Input: dimensioned drawing with shaded views. Units: mm. Origin: part minimum x, y, z. Round coordinates to 2 decimals unless told otherwise and drop trailing zeros. Loops run counter-clockwise (first coordinate to the right, second up) from the corner with the lowest first, then second, coordinate; pieces in that order, holes last. Notation, with made-up numbers: (-33.75, -26.75) - (-1.75, -26.75) arc R19 ccw to (-1.75, -12.75) - close; hole circle Ø7 at (62.25, 61.5). An arc over 180 degrees is marked (long way). Write each question's results on one line, items separated by ' | '.
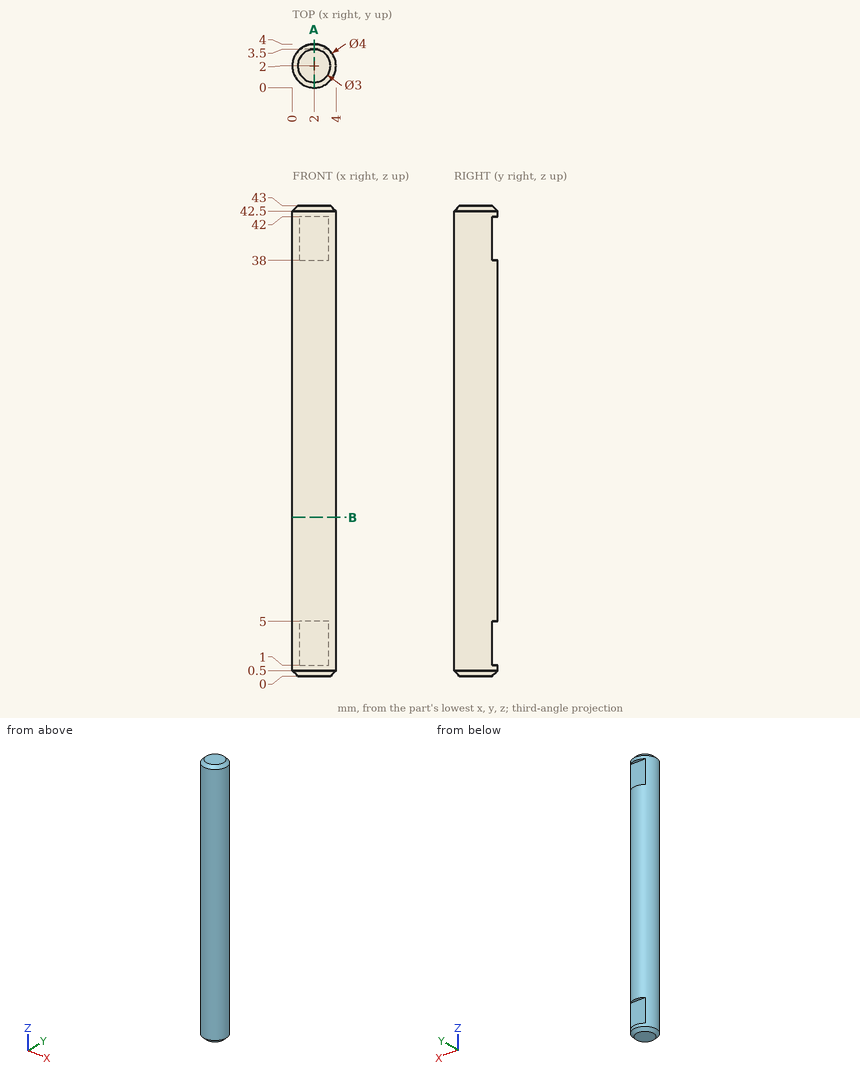
1. Line query: line 1 (Y direction, x = 2.1, z = 4); line 2 (X direction, y = 1.9, z = 32.5); line 3 (X direction, y = 1.1, z = 20). Output: solid intervals per line, ascending. Write a range as [from, to].
Answer:
line 1: [0, 3.5] | line 2: [0, 4] | line 3: [0.21, 3.79]
2. Contact query for a flat-ended pin moving along its axis: pin 1 (1.5 mm diameter, centred on y = 3.5, z = 12, fed in from +X). Output: stop coordinate, or through.
Answer:
pin 1: x = 3.85
3. Section query B-B, the plane z = 14.5. Output: boundary loops of the cut face in (x, y).
Answer:
outline: circle Ø4 at (2, 2)
4. Section query A-A, the plane x = 2. Output: boundary loops of the cut face in (y, z).
Answer:
outline: (0, 0.5) - (0.5, 0) - (3.5, 0) - (4, 0.5) - (4, 1) - (3.5, 1) - (3.5, 5) - (4, 5) - (4, 38) - (3.5, 38) - (3.5, 42) - (4, 42) - (4, 42.5) - (3.5, 43) - (0.5, 43) - (0, 42.5) - close
